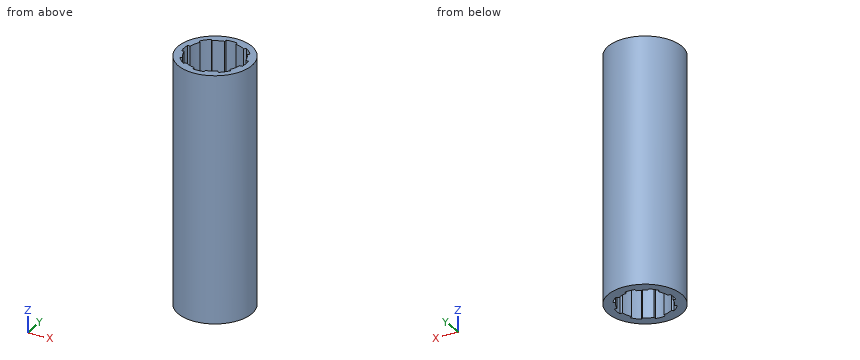
```python
from build123d import *

# Parameters (mm, degrees)
SKETCH_1_R          = 30
EXTRUDE_1_DEPTH     = 100
CUT_EXTRUDE_1_DEPTH = 80
CUT_EXTRUDE_START   = -80
CUT_EXTRUDE_2_DEPTH = 80


with BuildPart() as part:
    # 草图1 → 凸台-拉伸1 (new, symmetric)
    with BuildSketch(Plane.XY):
        with Locations(Location((0, 0, 0), (0, 0, 180))):
            Circle(SKETCH_1_R)
    extrude(amount=EXTRUDE_1_DEPTH, both=True)

    # 草图2 → 切除-拉伸1 (cut)
    with BuildSketch(Plane.XY.offset(100)):
        with BuildLine():
            Line((-4.5, 24.591665255), (-4.5, 22.555487137))
            ThreePointArc((-4.5, 22.555487137), (-8.801718944, 21.249229248), (-12.767157392, 19.131118423))
            Line((-12.767157392, 19.131118423), (-14.206952747, 20.570913778))
            ThreePointArc((-14.206952747, 20.570913778), (-17.67766953, 17.67766953), (-20.570913778, 14.206952747))
            Line((-20.570913778, 14.206952747), (-19.131118423, 12.767157392))
            ThreePointArc((-19.131118423, 12.767157392), (-21.249229248, 8.801718944), (-22.555487137, 4.5))
            Line((-22.555487137, 4.5), (-24.591665255, 4.5))
            ThreePointArc((-24.591665255, 4.5), (-25, 0), (-24.591665255, -4.5))
            Line((-24.591665255, -4.5), (-22.555487137, -4.5))
            ThreePointArc((-22.555487137, -4.5), (-21.249229248, -8.801718944), (-19.131118423, -12.767157392))
            Line((-19.131118423, -12.767157392), (-20.570913778, -14.206952747))
            ThreePointArc((-20.570913778, -14.206952747), (-17.67766953, -17.67766953), (-14.206952747, -20.570913778))
            Line((-14.206952747, -20.570913778), (-12.767157392, -19.131118423))
            ThreePointArc((-12.767157392, -19.131118423), (-8.801718944, -21.249229248), (-4.5, -22.555487137))
            Line((-4.5, -22.555487137), (-4.5, -24.591665255))
            ThreePointArc((-4.5, -24.591665255), (0, -25), (4.5, -24.591665255))
            Line((4.5, -24.591665255), (4.5, -22.555487137))
            ThreePointArc((4.5, -22.555487137), (8.801718944, -21.249229248), (12.767157392, -19.131118423))
            Line((12.767157392, -19.131118423), (14.206952747, -20.570913778))
            ThreePointArc((14.206952747, -20.570913778), (17.67766953, -17.67766953), (20.570913778, -14.206952747))
            Line((20.570913778, -14.206952747), (19.131118423, -12.767157392))
            ThreePointArc((19.131118423, -12.767157392), (21.249229248, -8.801718944), (22.555487137, -4.5))
            Line((22.555487137, -4.5), (24.591665255, -4.5))
            ThreePointArc((24.591665255, -4.5), (25, 0), (24.591665255, 4.5))
            Line((24.591665255, 4.5), (22.555487137, 4.5))
            ThreePointArc((22.555487137, 4.5), (21.249229248, 8.801718944), (19.131118423, 12.767157392))
            Line((19.131118423, 12.767157392), (20.570913778, 14.206952747))
            ThreePointArc((20.570913778, 14.206952747), (17.67766953, 17.67766953), (14.206952747, 20.570913778))
            Line((14.206952747, 20.570913778), (12.767157392, 19.131118423))
            ThreePointArc((12.767157392, 19.131118423), (8.801718944, 21.249229248), (4.5, 22.555487137))
            Line((4.5, 22.555487137), (4.5, 24.591665255))
            ThreePointArc((4.5, 24.591665255), (0, 25), (-4.5, 24.591665255))
        make_face()
    extrude(amount=-CUT_EXTRUDE_1_DEPTH, mode=Mode.SUBTRACT)

    # 草图3 → 切除-拉伸2 (cut)
    with BuildSketch(Plane(origin=(0, 0, -100), x_dir=(-1, 0, 0), z_dir=(0, 0, -1)).offset(CUT_EXTRUDE_START)):
        with BuildLine():
            Line((-4, 22.649503306), (-4, 20.615528128))
            ThreePointArc((-4, 20.615528128), (-8.03635208, 19.401470183), (-11.748952612, 17.405806862))
            Line((-11.748952612, 17.405806862), (-13.187190253, 18.844044503))
            ThreePointArc((-13.187190253, 18.844044503), (-16.263455967, 16.263455967), (-18.844044503, 13.187190253))
            Line((-18.844044503, 13.187190253), (-17.405806862, 11.748952612))
            ThreePointArc((-17.405806862, 11.748952612), (-19.401470183, 8.03635208), (-20.615528128, 4))
            Line((-20.615528128, 4), (-22.649503306, 4))
            ThreePointArc((-22.649503306, 4), (-23, 0), (-22.649503306, -4))
            Line((-22.649503306, -4), (-20.615528128, -4))
            ThreePointArc((-20.615528128, -4), (-19.401470183, -8.03635208), (-17.405806862, -11.748952612))
            Line((-17.405806862, -11.748952612), (-18.844044503, -13.187190253))
            ThreePointArc((-18.844044503, -13.187190253), (-16.263455967, -16.263455967), (-13.187190253, -18.844044503))
            Line((-13.187190253, -18.844044503), (-11.748952612, -17.405806862))
            ThreePointArc((-11.748952612, -17.405806862), (-8.03635208, -19.401470183), (-4, -20.615528128))
            Line((-4, -20.615528128), (-4, -22.649503306))
            ThreePointArc((-4, -22.649503306), (0, -23), (4, -22.649503306))
            Line((4, -22.649503306), (4, -20.615528128))
            ThreePointArc((4, -20.615528128), (8.03635208, -19.401470183), (11.748952612, -17.405806862))
            Line((11.748952612, -17.405806862), (13.187190253, -18.844044503))
            ThreePointArc((13.187190253, -18.844044503), (16.263455967, -16.263455967), (18.844044503, -13.187190253))
            Line((18.844044503, -13.187190253), (17.405806862, -11.748952612))
            ThreePointArc((17.405806862, -11.748952612), (19.401470183, -8.03635208), (20.615528128, -4))
            Line((20.615528128, -4), (22.649503306, -4))
            ThreePointArc((22.649503306, -4), (23, 0), (22.649503306, 4))
            Line((22.649503306, 4), (20.615528128, 4))
            ThreePointArc((20.615528128, 4), (19.401470183, 8.03635208), (17.405806862, 11.748952612))
            Line((17.405806862, 11.748952612), (18.844044503, 13.187190253))
            ThreePointArc((18.844044503, 13.187190253), (16.263455967, 16.263455967), (13.187190253, 18.844044503))
            Line((13.187190253, 18.844044503), (11.748952612, 17.405806862))
            ThreePointArc((11.748952612, 17.405806862), (8.03635208, 19.401470183), (4, 20.615528128))
            Line((4, 20.615528128), (4, 22.649503306))
            ThreePointArc((4, 22.649503306), (0, 23), (-4, 22.649503306))
        make_face()
    extrude(amount=CUT_EXTRUDE_2_DEPTH, mode=Mode.SUBTRACT)


solid = part.part
```
CAD build for the part. Positions are in the model's coordinates, mm. Round coordinates to 2 decimals unless told otherwise and drop trailing zeros. Order: outer loops, then holes, each group sorted by start corner. A loop starts at its lowest first (then second) coordinate and runs counter-clockwise, first axis right, second up. Notation, with made-up numbers: (38, 37) -> (81, 37) arc R16 cw to (81, 48) -> close; hole circle Ø3 at (22.5, -37.5). An arc over 180 degrees is marked (long way). Write item = value, one per line.
(1) Cut at B-B (x = 0). Write the cut outline in (y, z), plus the area to 3 significant figures.
Answers follow:
outline = (-30, -100) -> (-23, -100) -> (-23, -20) -> (23, -20) -> (23, -100) -> (30, -100) -> (30, 100) -> (25, 100) -> (25, 20) -> (-25, 20) -> (-25, 100) -> (-30, 100) -> close
area = 4,320 mm²
(2) Flat gauge pins, fed straight in: P1, Ø1, axis at x = 23.5, z = 74, coming from the +Y side; P2, Ø3, axis at x = -3, z = -3.5, coming from the +Y side; P3, Ø1, axis at y = 22.5, z = -34, coming from the -X side; P4, Ø23, axis at x = -8.5, y = 7, coming from the -Z side. Where does each tip first touch, or does it go through?
Answers follow:
P1 = 19.26
P2 = 29.96
P3 = -20.4
P4 = -100
(3) Drill centre lines: L1, parallel to X at y = 20.5, z = 59.5; L2, parallel to X at y = 10.5, z = 45; L3, parallel to Z at x = 13.5, y = -9. Where is each one in solid material? Low to high.
Answers follow:
L1 = -21.9 to -14.31, -14.14 to -10.43, 10.43 to 14.14, 14.31 to 21.9
L2 = -28.1 to -20.46, 20.46 to 28.1
L3 = -20 to 20
